Can you work these out from the model? Positions are in its coordinate system, mm. Give positions to 0.01 mm unless a question says otherwise; leave off trailing zeros. Use CSV: the item, a comma, the result in double quotes.
from build123d import *

# Parameters (mm, degrees)
SKETCH_1_W         = 300
SKETCH_1_H         = 115
EXTRUDE_1_DEPTH    = 12
HOLE_WIZARD_M6_1_D = 5
HOLE_WIZARD_M4_2_D = 3.3
HOLE_WIZARD_M5_1_D = 4.2
CHAMFER_1_SIZE     = 2


with BuildPart() as part:
    # 草图1 → 凸台-拉伸1 (new body)
    with BuildSketch(Plane.XY):
        Rectangle(SKETCH_1_W, SKETCH_1_H)
    extrude(amount=EXTRUDE_1_DEPTH)

    # M6 螺纹孔1 (through all)
    with Locations(Plane(origin=(0, 0, 0), x_dir=(-1, 0, 0), z_dir=(0, 0, -1))):
        with Locations((130, 19), (60, -19), (60, 19), (130, -19), (20, 19), (-50, -19), (-50, 19), (20, -19)):
            Hole(HOLE_WIZARD_M6_1_D / 2)

    # M4 螺纹孔2 (through all)
    with Locations(Plane.XY.offset(12)):
        with Locations((-144, 15), (-144, -2), (118, 15), (118, -2)):
            Hole(HOLE_WIZARD_M4_2_D / 2)

    # M5 螺纹孔1 (through all)
    with Locations(Plane(origin=(0, 0, 0), x_dir=(-1, 0, 0), z_dir=(0, 0, -1))):
        with Locations((110, 47.5), (70, 47.5)):
            Hole(HOLE_WIZARD_M5_1_D / 2)

    # 倒角1
    chamfer_1_edges = [part.edges().sort_by_distance(p)[0] for p in [
        (150, -57.5, 6),
        (-150, -57.5, 6),
        (-150, 57.5, 6),
        (150, 57.5, 6),
    ]]
    chamfer(chamfer_1_edges, length=CHAMFER_1_SIZE)


solid = part.part
Q1. I'm going to push flat-ended pins straight in: P1, Ø4, axis at x = 50, y = 19, coming from the -Z side; P2, Ø4.5, axis at x = -144, y = -2, coming from the +Z side. Where does each tip first touch, or does it pass through?
Model answer:
P1,"through"
P2,"z = 12"
Q2. If we mould it in two halves opening along Y, with no side actions, what happens to faces 1 (the flat face through (150, -1, 6)), 2 (the cylindrical face through (-58.66, 21.11, 6.08)), 3 (the flat face through (-2, 57.5, 6))? For each: released by +Y, released by -Y, zero draft, split by the parting line, or undercut.
Model answer:
face 1,"zero draft"
face 2,"undercut"
face 3,"released by +Y"
Q3. Please list where these lines run through material, in increasing order: L1, parallel to Y at x = 50, z = 3.5; L2, parallel to X at y = -19.5, z = 2; L3, parallel to X at y = 21, z = 9.75. Write a range as from..to.
Model answer:
L1,"-57.5..-21.5, -16.5..16.5, 21.5..57.5"
L2,"-150..-132.45, -127.55..-62.45, -57.55..-22.45, -17.55..47.55, 52.45..150"
L3,"-150..-131.5, -128.5..-61.5, -58.5..-21.5, -18.5..48.5, 51.5..150"
